CAD build for the part. Positions are in the model's coordinates, mm. A direction names the side the tool comes from. Round coordinates to 2 decimals unless told otherwise and drop trailing zeros. Write each loop counter-clockwise with the first axis right and the second up, starting at its lowest first coordinate (ties: lowest second). Pieces come first, ordered by that corner, then holes. Notation, with made-up numbers: (76, 20.5) -> (115, 20.5) arc R25 ccw to (115, 45.5) -> close; hole circle Ø2 at (-36.75, 27.5). An arc over 180 degrees is marked (long way). Put each result on its own line as item: value. Start each with the question number.
1. Pull direction Z, two halves, no side cores. Call faces 1 (the cylindrical face through (0.176, 87.725, 13.465)), 2 (the flat face through (0, 3, 16)), 3 (the flat face through (0, -10, 8)): pulls with the +Z half, pulls with the -Z half, needs draft (parallel to the pull), parting line crosses it, or undercut.
2. Flat gauge pins, fed straight in: P1, Ø1.8, axis at x = 3.5, z = 7.5, coming from the -Y side; P2, Ø9.5, axis at x = 0, y = 79.73, coming from the +Z side; P3, Ø3, axis at x = 4, z = 9, coming from the +Y side; P4, Ø6, axis at x = -3, z = 9, coming from the +Y side. Where does each tip first touch, or does it go through?
3. Drill centre lines: line 1 (Y direction, x = 0, z = 14.3); line 2 (Z direction, x = -0.75, y = 71); line 3 (Y direction, x = -1.5, z = 2.5). Where is each one in solid material? Low to high. Write a range as from..to.
4. Saw through at B-B on y = -13.5. List the corners of the cut face in (x, z), and give its area (3 significant figures).
5. 3-axis set-ups, long thin cutter, end or side, ignore diameter. For faces 4 (the flat face through (0, -47, 5)), 5 (the flat face through (0, 10, 8)), 6 (the cylindrical face through (-0.4, 82.7, 13.5)): which of +Z, -Z, +X, -X, +Y, -Y reach the whole face in a straight line?
6. Saw through at D-D on z = 7. List the corners of the cut face in (x, y), and give its area (3 significant figures).
7. Saw through at A-A on x = 0. List the corners of the cut face in (y, z).
8. Saw through at C-C on x = 6.25. List the corners of the cut face in (y, z), and give its area (3 significant figures).
from build123d import *

# Parameters (mm, degrees)
SKETCH1_R           = 3
BOSS_EXTRUDE1_DEPTH = 16
SKETCH2_W           = 6
SKETCH2_H           = 139.453359721
SKETCH2_H_2         = 146.546640279
CUT_EXTRUDE1_DEPTH  = 91.59784964


with BuildPart() as part:
    # Sketch1 → Boss-Extrude1 (new body)
    with BuildSketch(Plane.XY):
        with BuildLine():
            Line((-8, 79.726679861), (-8, -75.273320139))
            ThreePointArc((-8, -75.273320139), (0, -83.273320139), (8, -75.273320139))
            Line((8, -75.273320139), (8, 79.726679861))
            ThreePointArc((8, 79.726679861), (0, 87.726679861), (-8, 79.726679861))
        make_face()
        with Locations((0, 79.726679861)):
            Circle(SKETCH1_R, mode=Mode.SUBTRACT)
        with Locations((0, -75.273320139)):
            Circle(SKETCH1_R, mode=Mode.SUBTRACT)
    extrude(amount=BOSS_EXTRUDE1_DEPTH)

    # Sketch2 → Cut-Extrude1 (cut, through all)
    with BuildSketch(Plane(origin=(8, 0, 0), x_dir=(0, 0, -1), z_dir=(1, 0, 0))):
        with Locations((-8, 79.72667986)):
            Rectangle(SKETCH2_W, SKETCH2_H)
        with Locations((-8, -83.27332014)):
            Rectangle(SKETCH2_W, SKETCH2_H_2)
    extrude(amount=-CUT_EXTRUDE1_DEPTH, mode=Mode.SUBTRACT)


solid = part.part
Return value:
1. face 1: needs draft
1. face 2: pulls with the +Z half
1. face 3: undercut
2. P1: stops at y = -10
2. P2: stops at z = 16
2. P3: stops at y = 10
2. P4: stops at y = 87.69
3. line 1: y = -83.27..-78.27, -72.27..76.73, 82.73..87.73
3. line 2: z = 0..5, 11..16
3. line 3: y = -83.13..-77.87, -72.68..77.13, 82.32..87.58
4. outline: (-8, 0) -> (8, 0) -> (8, 5) -> (-8, 5) -> close; (-8, 11) -> (8, 11) -> (8, 16) -> (-8, 16) -> close
4. area: 160 mm^2
5. face 4: +X, -X, -Y
5. face 5: +X, -X, +Y
5. face 6: +Z, -Z
6. outline: (-8, -10) -> (8, -10) -> (8, 10) -> (-8, 10) -> close
6. area: 320 mm^2
7. outline: (-83.27, 0) -> (-78.27, 0) -> (-78.27, 5) -> (-83.27, 5) -> close; (-83.27, 11) -> (-78.27, 11) -> (-78.27, 16) -> (-83.27, 16) -> close; (-72.27, 0) -> (76.73, 0) -> (76.73, 5) -> (10, 5) -> (10, 11) -> (76.73, 11) -> (76.73, 16) -> (-72.27, 16) -> (-72.27, 11) -> (-10, 11) -> (-10, 5) -> (-72.27, 5) -> close; (82.73, 0) -> (87.73, 0) -> (87.73, 5) -> (82.73, 5) -> close; (82.73, 11) -> (87.73, 11) -> (87.73, 16) -> (82.73, 16) -> close
8. outline: (-80.27, 0) -> (84.72, 0) -> (84.72, 5) -> (10, 5) -> (10, 11) -> (84.72, 11) -> (84.72, 16) -> (-80.27, 16) -> (-80.27, 11) -> (-10, 11) -> (-10, 5) -> (-80.27, 5) -> close
8. area: 1,770 mm^2
